from build123d import *

# Parameters (mm, degrees)
SKETCH_1_W                   = 40
SKETCH_1_H                   = 25
EXTRUDE_1_DEPTH              = 15
SKETCH_9_W                   = 40
SKETCH_9_H                   = 8.2
EXTRUDE_3_DEPTH              = 3
HOLE_WIZARD_M6_2_D           = 6.6
HOLE_WIZARD_M6_2_CBORE_D     = 11
HOLE_WIZARD_M6_2_CBORE_DEPTH = 6.4
SKETCH_12_R                  = 3
CUT_EXTRUDE_3_DEPTH          = 51.487622245
CHAMFER_2_SIZE               = 0.5
CHAMFER_3_SIZE               = 2


with BuildPart() as part:
    # 草图1 → 凸台-拉伸1 (new body)
    with BuildSketch(Plane.XY):
        with Locations((20, 12.5)):
            Rectangle(SKETCH_1_W, SKETCH_1_H)
    extrude(amount=EXTRUDE_1_DEPTH)

    # 草图9 → 凸台-拉伸3 (add)
    with BuildSketch(Plane(origin=(0, 0, 0), x_dir=(-1, 0, 0), z_dir=(0, 0, -1))):
        with Locations((-20, 12.5)):
            Rectangle(SKETCH_9_W, SKETCH_9_H)
    extrude(amount=EXTRUDE_3_DEPTH)

    # M6 六角凹头螺钉的柱形沉头孔2 (through all)
    with Locations(Plane.XY.offset(15)):
        with Locations((10, 12.5)):
            CounterBoreHole(HOLE_WIZARD_M6_2_D / 2, HOLE_WIZARD_M6_2_CBORE_D / 2, HOLE_WIZARD_M6_2_CBORE_DEPTH)

    # 草图12 → 切除-拉伸3 (cut, through all)
    with BuildSketch(Plane.XY.offset(15)):
        with Locations((32.5, 12.5)):
            Circle(SKETCH_12_R)
    extrude(amount=-CUT_EXTRUDE_3_DEPTH, mode=Mode.SUBTRACT)

    # 倒角2
    chamfer_2_edges = [part.edges().sort_by_distance(p)[0] for p in [
        (29.5, 12.5, 15),
    ]]
    chamfer(chamfer_2_edges, length=CHAMFER_2_SIZE)

    # 倒角3
    chamfer_3_edges = [part.edges().sort_by_distance(p)[0] for p in [
        (40, 0, 7.5),
        (0, 0, 7.5),
        (0, 25, 7.5),
        (40, 25, 7.5),
    ]]
    chamfer(chamfer_3_edges, length=CHAMFER_3_SIZE)


solid = part.part
Could you check a few things on this model? Use its own coordinates, in mm. A direction names the side the tool comes from. Coordinates: 2 decimals unless noted, no trailing zeros. Loops run counter-clockwise (first coordinate to the right, second up) from the corner with the lowest first, then second, coordinate; pieces in that order, holes last. Notation, with made-up numbers: (24, 53) -> (52, 53) arc R17 ccw to (52, 65) -> close; hole circle Ø7 at (62, 12). An arc over 180 degrees is marked (long way). Answer in a Markdown table with one row per item.
(1) For faces 4 (the face through (20, 13, 15)), 5 (the face through (12.5, 7.6, 11.8)), 6 (the face through (20, 21, 0)), 7 (the face through (20, 8.4, -1)), 8 (the face through (39, 1, 7)), which set-ups out of +Z, -Z, +X, -X, +Y, -Y let a thin tool reach every point of the face, with its end or its side?
Results found:
| item | result |
|---|---|
| face 4 | +Z, +X, -X, +Y, -Y |
| face 5 | +Z |
| face 6 | -Z, +X, -X, +Y |
| face 7 | -Z, +X, -X, -Y |
| face 8 | +Z, -Z, +X, -Y |
(2) Imagine slicing it at D-D (x = 4). List the corners of the cut face in (y, z) for me, plus the area to 3 significant figures.
Results found:
| item | result |
|---|---|
| outline | (0, 0) -> (8.4, 0) -> (8.4, -3) -> (16.6, -3) -> (16.6, 0) -> (25, 0) -> (25, 15) -> (0, 15) -> close |
| area | 400 mm^2 |
(3) If I drill on probe 1 along Y at (x, z) = (10, 12); probe 2 along Y at (x, z) = (10, 2); probe 3 along Z at (x, y) = (33.5, 5), over which ranges is the centre line in solid material (lowest first)?
Results found:
| item | result |
|---|---|
| probe 1 | y = 0 to 7, 18 to 25 |
| probe 2 | y = 0 to 9.2, 15.8 to 25 |
| probe 3 | z = 0 to 15 |
(4) Imagine slicing it at B-B (y = 12.5). List the corners of the cut face in (x, z) for me.
Results found:
| item | result |
|---|---|
| outline | (0, -3) -> (6.7, -3) -> (6.7, 8.6) -> (4.5, 8.6) -> (4.5, 15) -> (0, 15) -> close; (13.3, -3) -> (29.5, -3) -> (29.5, 14.5) -> (29, 15) -> (15.5, 15) -> (15.5, 8.6) -> (13.3, 8.6) -> close; (35.5, -3) -> (40, -3) -> (40, 15) -> (36, 15) -> (35.5, 14.5) -> close |
(5) Thinking about a two-plate mould opening in Y: for faces 1 (the face through (14, 13, 8.6)), 2 (the face through (1, 1, 7)), 3 (the face through (39, 24, 7)), which applies, released by +Y, released by -Y, zero draft, split by the parting line, or undercut?
Results found:
| item | result |
|---|---|
| face 1 | undercut |
| face 2 | released by -Y |
| face 3 | released by +Y |
(6) Will these pins go through, and if not, where does the flat tip stop? pin 1 Ø2 at (x, y) = (23.5, 3) entering from -Z; pin 2 Ø0.9 at (x, z) = (27, -1.5) entering from +Y.
Results found:
| item | result |
|---|---|
| pin 1 | stops at z = 0 |
| pin 2 | stops at y = 16.6 |
(7) Imagine slicing it at C-C (z = 9.25). List the corners of the cut face in (x, y) for me, plus the area to 3 significant figures.
Results found:
| item | result |
|---|---|
| outline | (0, 2) -> (2, 0) -> (38, 0) -> (40, 2) -> (40, 23) -> (38, 25) -> (2, 25) -> (0, 23) -> close; hole circle Ø11 at (10, 12.5); hole circle Ø6 at (32.5, 12.5) |
| area | 869 mm^2 |
(8) Imagine slicing it at A-A (x = 10). List the corners of the cut face in (y, z) for me.
Results found:
| item | result |
|---|---|
| outline | (0, 0) -> (8.4, 0) -> (8.4, -3) -> (9.2, -3) -> (9.2, 8.6) -> (7, 8.6) -> (7, 15) -> (0, 15) -> close; (15.8, -3) -> (16.6, -3) -> (16.6, 0) -> (25, 0) -> (25, 15) -> (18, 15) -> (18, 8.6) -> (15.8, 8.6) -> close |
